Could you check a few things on this model? Use its own coordinates, in mm. Face numbers are marked on the shaded views. A direction names the side the tool comes from. Give positions to 0.01 mm unless a question says otherwise; leave off trailing zeros. Write each loop counter-clockwise with the first axis right and the second up, starting at its lowest first coordinate (ties: lowest second). Pieces come first, ordered by that corner, then holes. Notation, with made-up numbers: (42.5, 71.25) - (50.5, 71.25) arc R32 ccw to (50.5, 109.25) - close; hole circle Ø7 at (22, 74.5). An arc over 180 degrees is marked (long way). Answer as a JSON object with one key per item and string values. Group by question number.
```python
from build123d import *

# Parameters (mm, degrees)
EXTRUDE_1_DEPTH         = 7.5
CHAMFER_1_SIZE          = 5
HOLE_WIZARD_5_5_5_5_1_D = 5.5
HOLE_WIZARD_5_5_5_5_2_D = 5.5


with BuildPart() as part:
    # 草图1 → 凸台-拉伸1 (new, symmetric)
    with BuildSketch(Plane(origin=(0, 0, 0), x_dir=(1, 0, 0), z_dir=(0, 1, 0))):
        Polygon((30, 0), (0, 0), (0, -45), (-15, -45), (-15, 15), (30, 15), align=None)
    extrude(amount=EXTRUDE_1_DEPTH, both=True)

    # 倒角1
    chamfer_1_edges = [part.edges().sort_by_distance(p)[0] for p in [
        (30, 0, 0),
        (0, 0, 45),
    ]]
    chamfer(chamfer_1_edges, length=CHAMFER_1_SIZE)

    # Ø5.5 (5.5) 直径孔1 (through all)
    with Locations(Plane(origin=(0, 0, 0), x_dir=(0, 0, -1), z_dir=(1, 0, 0))):
        with Locations((-35, 0), (-15, 0)):
            Hole(HOLE_WIZARD_5_5_5_5_1_D / 2)

    # Ø5.5 (5.5) 直径孔2 (through all)
    with Locations(Plane.XY):
        with Locations((15, 0)):
            Hole(HOLE_WIZARD_5_5_5_5_2_D / 2)


solid = part.part
```
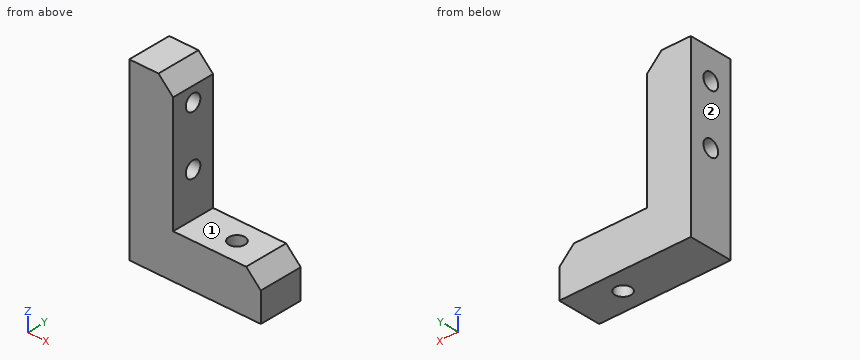
(1) For the marked faces 1 and 2, which set-ups out of +Z, -Z, +X, -X, +Y, -Y let a thin tool reach every point of the face, with its end or its side?
(2) I want a section at C-C, the plane y = 0. Please give me the cut outline in (x, z), and give its area (3 significant figures).
(3) I want a section at D-D, the plane y = -3.5. Please give me the cut outline in (x, z).
(4) I need wall thicknesses on L1, parallel to Z at x = -11, y = 1.75; L2, parallel to Y at x = -6.75, z = 15; L3, parallel to Z at x = -13, y = 2. Which ranges of each line are inside material? Lowest first, please.
(5) I want a section at A-A, the plane z = 15. Please give me the cut outline in (x, y), and give its area (4 significant figures).
(6) I want a section at B-B, the plane x = 15. Please give me the cut outline in (y, z).
(7) Will these pins go through, and if not, where does the flat tip stop? P1, Ø4.5, axis at x = 8.5, y = -1, coming from the +Z side; P2, Ø4.5, axis at y = 2, z = 24.5, coming from the +X side.
Entries:
{
 "1": {"face 1": "+Z, +X, +Y, -Y", "face 2": "+Z, -Z, -X, +Y, -Y"},
 "2": {"outline": "(-15, -15) - (12.25, -15) - (12.25, 0) - (0, 0) - (0, 12.25) - (-15, 12.25) - close; (-15, 17.75) - (0, 17.75) - (0, 32.25) - (-15, 32.25) - close; (-15, 37.75) - (0, 37.75) - (0, 40) - (-5, 45) - (-15, 45) - close; (17.75, -15) - (30, -15) - (30, -5) - (25, 0) - (17.75, 0) - close", "area": "1,080 mm^2"},
 "3": {"outline": "(-15, -15) - (30, -15) - (30, -5) - (25, 0) - (0, 0) - (0, 40) - (-5, 45) - (-15, 45) - close"},
 "4": {"L1": "-15 to 12.88, 17.12 to 32.88, 37.12 to 45", "L2": "-7.5 to -2.75, 2.75 to 7.5", "L3": "-15 to 13.11, 16.89 to 33.11, 36.89 to 45"},
 "5": {"outline": "(-15, -7.5) - (0, -7.5) - (0, -2.75) - (-15, -2.75) - close; (-15, 2.75) - (0, 2.75) - (0, 7.5) - (-15, 7.5) - close", "area": "142.5 mm^2"},
 "6": {"outline": "(-7.5, -15) - (-2.75, -15) - (-2.75, 0) - (-7.5, 0) - close; (2.75, -15) - (7.5, -15) - (7.5, 0) - (2.75, 0) - close"},
 "7": {"P1": "z = 0", "P2": "x = 0"}
}
